Read the model definition and answer for the solid it produces. Units are mm, in the model's axes. Face numbers are marked on the shaded views. A direction names the side the tool comes from. Give positions to 0.01 mm unless a question says otherwise; leave off trailing zeros. Order: outer loops, then holes, each group sorted by start corner. A loop starts at its lowest first (then second) coordinate and runs counter-clockwise, first axis right, second up. Notation, with made-up numbers: (66, 14.5) -> (110, 14.5) arc R6 cw to (110, 18.5) -> close; hole circle Ø10 at (68, 52). An arc over 180 degrees is marked (long way). Use one line per item in the form item = value.
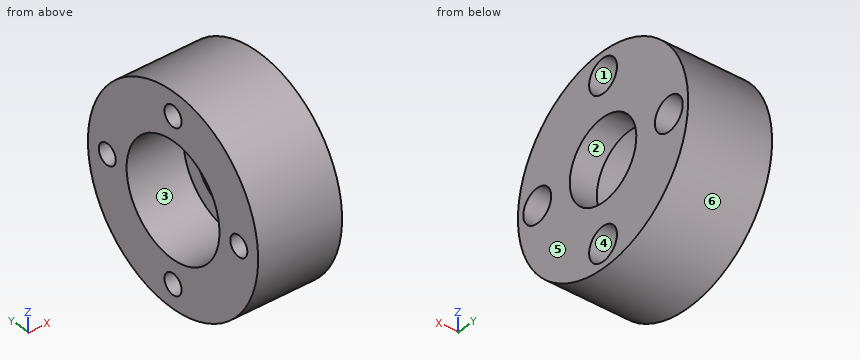
```python
from build123d import *

# Parameters (mm, degrees)
HOLE_SIZE_PER_SOCKET_HEAD_CAP_SCREW_TYPE_D           = 11
HOLE_SIZE_PER_SOCKET_HEAD_CAP_SCREW_TYPE_CBORE_D     = 18
HOLE_SIZE_PER_SOCKET_HEAD_CAP_SCREW_TYPE_CBORE_DEPTH = 20


with BuildPart() as part:
    # Sketch1 → Revolve1 (revolve)
    with BuildSketch(Plane.XY, mode=Mode.PRIVATE) as revolve1_sk:
        Polygon((48.914797255, 21.5), (63.414797255, 21.5), (63.414797255, 55), (18.414797255, 55), (18.414797255, 30), (48.914797255, 30), align=None)
    revolve(revolve1_sk.sketch.rotate(Axis((0, 0, 0), (1, 0, 0)), 90), axis=Axis((0, 0, 0), (1, 0, 0)))

    # Hole size per socket head cap screw type1 (through all)
    with Locations(Plane(origin=(63.414797255, 0, 0), x_dir=(0, 0, -1), z_dir=(1, 0, 0))):
        with Locations((0, 42.5), (0, -42.5), (-42.5, 0), (42.5, 0)):
            CounterBoreHole(HOLE_SIZE_PER_SOCKET_HEAD_CAP_SCREW_TYPE_D / 2, HOLE_SIZE_PER_SOCKET_HEAD_CAP_SCREW_TYPE_CBORE_D / 2, HOLE_SIZE_PER_SOCKET_HEAD_CAP_SCREW_TYPE_CBORE_DEPTH)


solid = part.part
```
Item 1: The part is cut by section A-A on y = 0. Give the vertices of the cut face in (x, z).
Checks:
outline = (18.41, -55) -> (63.41, -55) -> (63.41, -51.5) -> (43.41, -51.5) -> (43.41, -48) -> (18.41, -48) -> close; (18.41, -37) -> (43.41, -37) -> (43.41, -33.5) -> (63.41, -33.5) -> (63.41, -21.5) -> (48.91, -21.5) -> (48.91, -30) -> (18.41, -30) -> close; (18.41, 30) -> (48.91, 30) -> (48.91, 21.5) -> (63.41, 21.5) -> (63.41, 33.5) -> (43.41, 33.5) -> (43.41, 37) -> (18.41, 37) -> close; (18.41, 48) -> (43.41, 48) -> (43.41, 51.5) -> (63.41, 51.5) -> (63.41, 55) -> (18.41, 55) -> close
Item 2: The part is cut by section B-B on x = 35. Give the vertices of the cut face in (y, z).
Checks:
outline = circle Ø110 at (0, 0); hole circle Ø11 at (-42.5, 0); hole circle Ø60 at (0, 0); hole circle Ø11 at (0, -42.5); hole circle Ø11 at (0, 42.5); hole circle Ø11 at (42.5, 0)
Item 3: The part is cut by section D-D on y = -11. Give the vertices of the cut face in (x, z).
Checks:
outline = (18.41, -53.89) -> (63.41, -53.89) -> (63.41, -18.47) -> (48.91, -18.47) -> (48.91, -27.91) -> (18.41, -27.91) -> close; (18.41, 27.91) -> (48.91, 27.91) -> (48.91, 18.47) -> (63.41, 18.47) -> (63.41, 53.89) -> (18.41, 53.89) -> close
Item 4: Which of the six approach directions +Z, -Z, +X, -X, +Y, -Y give full straight-line access (tool end or side, diameter ignored) to the marked faces 1, 2 and 3?
Checks:
face_1 = +X
face_2 = +X, -X
face_3 = -X
Item 5: Given pin 1 Ø4 at (x, y) = (48.5, 28.5) entering from -Z; pin 2 Ø1.5 at (x, y) = (56, 31.5) entering from +Z; pin 3 Ø14.5 at (y, z) = (42.5, 0) entering from +X, each flat-ended and moving along its own axis, determine where each tip first touches the part or whether it passes through.
Checks:
pin_1 = -48.19
pin_2 = 45.6
pin_3 = 43.41
Item 6: The part is cut by section C-C on z = -0.5. Give the vertices of the cut face in (x, y).
Checks:
outline = (18.41, -55) -> (63.41, -55) -> (63.41, -51.49) -> (43.41, -51.49) -> (43.41, -47.98) -> (18.41, -47.98) -> close; (18.41, -37.02) -> (43.41, -37.02) -> (43.41, -33.51) -> (63.41, -33.51) -> (63.41, -21.49) -> (48.91, -21.49) -> (48.91, -30) -> (18.41, -30) -> close; (18.41, 30) -> (48.91, 30) -> (48.91, 21.49) -> (63.41, 21.49) -> (63.41, 33.51) -> (43.41, 33.51) -> (43.41, 37.02) -> (18.41, 37.02) -> close; (18.41, 47.98) -> (43.41, 47.98) -> (43.41, 51.49) -> (63.41, 51.49) -> (63.41, 55) -> (18.41, 55) -> close
Item 7: Straight lines are drawn through the part: L1, parallel to Y at x = 29.75, z = 0; L2, parallel to Y at x = 52.75, z = 0; L3, parallel to Z at x = 35, y = -5. For each, find the intervals that lie inside material, in ascending order. Write a range as from..to.
Checks:
L1 = -55..-48, -37..-30, 30..37, 48..55
L2 = -55..-51.5, -33.5..-21.5, 21.5..33.5, 51.5..55
L3 = -54.77..-44.79, -40.21..-29.58, 29.58..40.21, 44.79..54.77
Item 8: Determine the mould class of the marked faces 4, 5 and 6 for opening direction Z: +Z half, -Z half, draft (parallel to the pull), parting line (faces both ways), or undercut.
Checks:
face_4 = undercut
face_5 = draft
face_6 = parting line
